from build123d import *

# Parameters (mm, degrees)
SKETCH_1_W          = 1148
SKETCH_1_H          = 125
EXTRUDE_1_DEPTH     = 15
SHELL_1_T           = -2
SKETCH_2_W          = 1148
SKETCH_2_H          = 125
SKETCH_2_W_2        = 1132
SKETCH_2_H_2        = 109
EXTRUDE_2_DEPTH     = 2
SKETCH_3_W          = 120
SKETCH_3_H          = 30
CUT_EXTRUDE_1_DEPTH = 10


with BuildPart() as part:
    # 草图1 → 凸台-拉伸1 (new body)
    with BuildSketch(Plane.XY):
        with Locations((574, 62.5)):
            Rectangle(SKETCH_1_W, SKETCH_1_H)
    extrude(amount=EXTRUDE_1_DEPTH)

    # 抽壳1
    shell_1_openings = [part.faces().sort_by_distance(p)[0] for p in [
        (574, 62.5, 15),
    ]]
    offset(amount=SHELL_1_T, openings=shell_1_openings, kind=Kind.INTERSECTION)

    # 草图2 → 凸台-拉伸2 (add)
    with BuildSketch(Plane.XY.offset(15)):
        with Locations((574, 62.5)):
            Rectangle(SKETCH_2_W, SKETCH_2_H)
        with Locations((574, 62.5)):
            Rectangle(SKETCH_2_W_2, SKETCH_2_H_2, mode=Mode.SUBTRACT)
    extrude(amount=-EXTRUDE_2_DEPTH)

    # 草图3 → 切除-拉伸1 (cut)
    with BuildSketch(Plane(origin=(0, 0, 0), x_dir=(-1, 0, 0), z_dir=(0, 0, -1))):
        with Locations((-574, 80)):
            Rectangle(SKETCH_3_W, SKETCH_3_H)
    extrude(amount=-CUT_EXTRUDE_1_DEPTH, mode=Mode.SUBTRACT)


solid = part.part
Could you check a few things on this model? Use its own coordinates, in mm. Round coordinates to 2 decimals unless told otherwise and drop trailing zeros. Write each loop counter-clockwise with the first axis right and the second up, starting at its lowest first coordinate (ties: lowest second). Pieces come first, ordered by that corner, then holes. Notation, with made-up numbers: (36.5, -22.5) - (73.5, -22.5) arc R21 ccw to (73.5, -17.5) - close; hole circle Ø7 at (-22, -23). An arc over 180 degrees is marked (long way). Use a Markdown table: item, result.
Q1. I want a section at B-B (y = 35). List the corners of the cut face in (x, z) for me.
Output values:
| item | result |
|---|---|
| outline | (0, 0) - (1148, 0) - (1148, 15) - (1140, 15) - (1140, 13) - (1146, 13) - (1146, 2) - (2, 2) - (2, 13) - (8, 13) - (8, 15) - (0, 15) - close |
Q2. Please list where these lines run through material, in increasing order: L1, parallel to Y at x = 513, z = 8.5; L2, parallel to X at y = 91, z = 8; L3, parallel to X at y = 40, z = 13.25.
Output values:
| item | result |
|---|---|
| L1 | 0 to 2, 123 to 125 |
| L2 | 0 to 2, 1146 to 1148 |
| L3 | 0 to 8, 1140 to 1148 |
Q3. I want a section at A-A (z = 9). List the corners of the cut face in (x, y) for me.
Output values:
| item | result |
|---|---|
| outline | (0, 0) - (1148, 0) - (1148, 125) - (0, 125) - close; hole (2, 2) - (1146, 2) - (1146, 123) - (2, 123) - close |
Q4. For pin 1 (6 mm diameter, centred on x = 555, y = 21, fed in from +Z), with a flat end and sliding along its axis, tell me the tip position at first contact or that it passes through.
Output values:
| item | result |
|---|---|
| pin 1 | z = 2 |
Q5. I want a section at C-C (x = 891). List the corners of the cut face in (y, z) for me.
Output values:
| item | result |
|---|---|
| outline | (0, 0) - (125, 0) - (125, 15) - (117, 15) - (117, 13) - (123, 13) - (123, 2) - (2, 2) - (2, 13) - (8, 13) - (8, 15) - (0, 15) - close |
Q6. Thinking about a two-plate mould opening in Y: for faces 1 (the flat face through (571, 5, 13)), 2 (the flat face through (571, 118, 15)), which applies, released by +Y, released by -Y, zero draft, split by the parting line, or undercut?
Output values:
| item | result |
|---|---|
| face 1 | undercut |
| face 2 | zero draft |
